```python
from build123d import *

# Parameters (mm, degrees)
SKETCH_1_R                  = 1.6
SKETCH_1_R_2                = 20
EXTRUDE_1_DEPTH             = 3
HOLE_WIZARD_M3_1_AT_2_COUNT = 2
HOLE_WIZARD_M3_1_AT_2_PITCH = 25
HOLE_WIZARD_M3_1_AT_3_COUNT = 2
HOLE_WIZARD_M3_1_AT_3_PITCH = 43.301270189
HOLE_WIZARD_M3_1_AT_4_COUNT = 2
HOLE_WIZARD_M3_1_AT_4_PITCH = 50
HOLE_WIZARD_M3_1_AT_5_COUNT = 2
HOLE_WIZARD_M3_1_AT_5_PITCH = 43.301270189
HOLE_WIZARD_M3_1_AT_6_COUNT = 2
HOLE_WIZARD_M3_1_AT_6_PITCH = 25
SKETCH_3_R                  = 1.6
CUT_EXTRUDE_1_DEPTH         = 10
CUT_EXTRUDE_2_DEPTH         = 10
FILLET_1_R                  = 2


with BuildPart() as part:
    # 草图1 → 凸台-拉伸1 (new body)
    with BuildSketch(Plane(origin=(0, 0, 0), x_dir=(1, 0, 0), z_dir=(0, 1, 0))):
        with BuildLine():
            Line((-63.2, 35), (0, 35))
            Line((0, 35), (0, -35))
            Line((0, -35), (-63.2, -35))
            ThreePointArc((-63.2, -35), (-98.2, 0), (-63.2, 35))
        make_face()
        with Locations(Location((-63.2, 25, 0), (0, 0, 270))):
            Circle(SKETCH_1_R, mode=Mode.SUBTRACT)
        with Locations(Location((-41.549364905, 12.5, 0), (0, 0, 270))):
            Circle(SKETCH_1_R, mode=Mode.SUBTRACT)
        with Locations(Location((-41.549364905, -12.5, 0), (0, 0, 270))):
            Circle(SKETCH_1_R, mode=Mode.SUBTRACT)
        with Locations(Location((-63.2, -25, 0), (0, 0, 270))):
            Circle(SKETCH_1_R, mode=Mode.SUBTRACT)
        with Locations(Location((-84.850635095, -12.5, 0), (0, 0, 270))):
            Circle(SKETCH_1_R, mode=Mode.SUBTRACT)
        with Locations(Location((-84.850635095, 12.5, 0), (0, 0, 270))):
            Circle(SKETCH_1_R, mode=Mode.SUBTRACT)
        with Locations(Location((-63.2, 0, 0), (0, 0, 270))):
            Circle(SKETCH_1_R_2, mode=Mode.SUBTRACT)
        with Locations(Location((-25, 20, 0), (0, 0, 270))):
            Circle(SKETCH_1_R, mode=Mode.SUBTRACT)
        with Locations(Location((-5, 20, 0), (0, 0, 270))):
            Circle(SKETCH_1_R, mode=Mode.SUBTRACT)
        with Locations(Location((-5, -20, 0), (0, 0, 270))):
            Circle(SKETCH_1_R, mode=Mode.SUBTRACT)
        with Locations(Location((-25, -20, 0), (0, 0, 270))):
            Circle(SKETCH_1_R, mode=Mode.SUBTRACT)
    extrude(amount=EXTRUDE_1_DEPTH)

    # 草图2 → M3 六角凹锥坑螺钉的锥形沉头孔1 (revolve, cut)
    with BuildSketch(Plane(origin=(-63.2, 3, -25), x_dir=(0, 0, 1), z_dir=(1, 0, 0))):
        Polygon((0, 0), (0, 3), (1.6, 3), (1.6, 1.76), (3.36, 0), align=None)
    hole_wizard_m3_1 = revolve(axis=Axis((-63.2, 9.35, -25), (0, -1, 0)), mode=Mode.SUBTRACT)

    # M3 六角凹锥坑螺钉的锥形沉头孔1 at 2: M3 六角凹锥坑螺钉的锥形沉头孔1 ×2
    with Locations(*[Vector(0.8660254037844387, 0, 0.5) * (i * HOLE_WIZARD_M3_1_AT_2_PITCH) for i in range(1, HOLE_WIZARD_M3_1_AT_2_COUNT)]):
        add(hole_wizard_m3_1, mode=Mode.SUBTRACT)

    # M3 六角凹锥坑螺钉的锥形沉头孔1 at 3: M3 六角凹锥坑螺钉的锥形沉头孔1 ×2
    with Locations(*[Vector(0.5000000000000001, 0, 0.8660254037844386) * (i * HOLE_WIZARD_M3_1_AT_3_PITCH) for i in range(1, HOLE_WIZARD_M3_1_AT_3_COUNT)]):
        add(hole_wizard_m3_1, mode=Mode.SUBTRACT)

    # M3 六角凹锥坑螺钉的锥形沉头孔1 at 4: M3 六角凹锥坑螺钉的锥形沉头孔1 ×2
    with Locations(*[(0, 0, i * HOLE_WIZARD_M3_1_AT_4_PITCH) for i in range(1, HOLE_WIZARD_M3_1_AT_4_COUNT)]):
        add(hole_wizard_m3_1, mode=Mode.SUBTRACT)

    # M3 六角凹锥坑螺钉的锥形沉头孔1 at 5: M3 六角凹锥坑螺钉的锥形沉头孔1 ×2
    with Locations(*[Vector(-0.49999999999999983, 0, 0.8660254037844388) * (i * HOLE_WIZARD_M3_1_AT_5_PITCH) for i in range(1, HOLE_WIZARD_M3_1_AT_5_COUNT)]):
        add(hole_wizard_m3_1, mode=Mode.SUBTRACT)

    # M3 六角凹锥坑螺钉的锥形沉头孔1 at 6: M3 六角凹锥坑螺钉的锥形沉头孔1 ×2
    with Locations(*[Vector(-0.8660254037844388, 0, 0.4999999999999997) * (i * HOLE_WIZARD_M3_1_AT_6_PITCH) for i in range(1, HOLE_WIZARD_M3_1_AT_6_COUNT)]):
        add(hole_wizard_m3_1, mode=Mode.SUBTRACT)

    # 草图3 → 切除-拉伸1 (cut)
    with BuildSketch(Plane(origin=(0, 3, 0), x_dir=(1, 0, 0), z_dir=(0, 1, 0))):
        with Locations(Location((-31.7, 0, 0), (0, 0, 270))):
            Circle(SKETCH_3_R)
        with Locations(Location((-47.45, -27.279800219, 0), (0, 0, 270))):
            Circle(SKETCH_3_R)
        with Locations(Location((-78.95, -27.279800219, 0), (0, 0, 270))):
            Circle(SKETCH_3_R)
        with Locations(Location((-94.7, 0, 0), (0, 0, 270))):
            Circle(SKETCH_3_R)
        with Locations(Location((-78.95, 27.279800219, 0), (0, 0, 270))):
            Circle(SKETCH_3_R)
        with Locations(Location((-47.45, 27.279800219, 0), (0, 0, 270))):
            Circle(SKETCH_3_R)
    extrude(amount=-CUT_EXTRUDE_1_DEPTH, mode=Mode.SUBTRACT)

    # 草图4 → 切除-拉伸2 (cut)
    with BuildSketch(Plane(origin=(0, 3, 0), x_dir=(1, 0, 0), z_dir=(0, 1, 0))):
        Polygon((-23.5, 13.645898034), (-23.5, -13.645898034), (-16.677050983, 0), align=None)
        Polygon((-15, -3.354101966), (-22.572949017, -18.5), (-7.427050983, -18.5), align=None)
        Polygon((-7.427050983, 18.5), (-22.572949017, 18.5), (-15, 3.354101966), align=None)
        Polygon((-13.322949017, 0), (-6.5, -13.645898034), (-6.5, 13.645898034), align=None)
    extrude(amount=-CUT_EXTRUDE_2_DEPTH, mode=Mode.SUBTRACT)

    # 圆角1
    fillet_1_edges = [part.edges().sort_by_distance(p)[0] for p in [
        (-22.572949017, 1.5, 18.5),
        (-15, 1.5, 3.354101966),
        (-7.427050983, 1.5, 18.5),
        (-22.572949017, 1.5, -18.5),
        (-7.427050983, 1.5, -18.5),
        (-15, 1.5, -3.354101966),
        (-13.322949017, 1.5, 0),
        (-6.5, 1.5, -13.645898034),
        (-6.5, 1.5, 13.645898034),
        (-23.5, 1.5, 13.645898034),
        (-23.5, 1.5, -13.645898034),
        (-16.677050983, 1.5, 0),
        (0, 1.5, -35),
        (0, 1.5, 35),
    ]]
    fillet(fillet_1_edges, radius=FILLET_1_R)


solid = part.part
```
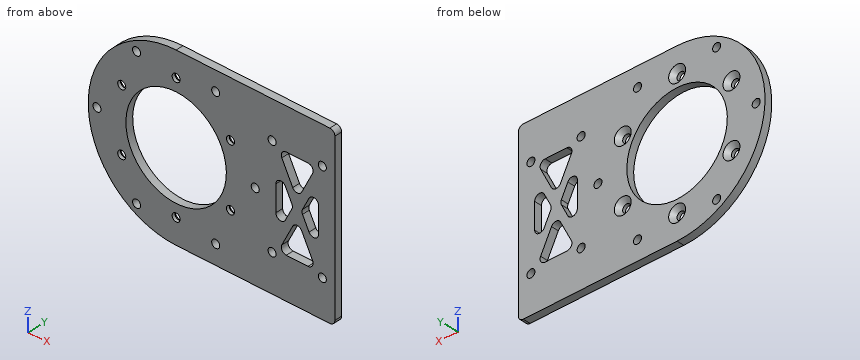
Check sheet for the modelled part. Datum: model origin and axes. Units: mm. Give positions to 0.01 mm unless a question says otherwise; leave off trailing zeros. Order: outer loops, then holes, each group sorted by start corner. A loop starts at its lowest first (then second) coordinate and runs counter-clockwise, first axis right, second up. Notation, with made-up numbers: (71, 17) -> (98, 17) arc R22 cw to (98, 47) -> close; hole circle Ø5 at (-32, -36). An arc over 180 degrees is marked (long way). Return JSON: item names as keys, results as strings.
1. Cross-section at B-B, the plane z = -17. Record the cut outline in (x, y).
From the geometry:
{"outline": "(-93.79, 0) -> (-73.74, 0) -> (-73.74, 3) -> (-93.79, 3) -> close; (-52.66, 0) -> (-21.27, 0) -> (-21.27, 3) -> (-52.66, 3) -> close; (-8.73, 0) -> (0, 0) -> (0, 3) -> (-8.73, 3) -> close"}
2. Material ranges on probe 1 along X at (y, z) = (2.4, 0); probe 2 along X at (y, z) = (2.8, 17); probe 3 along Z at (x, y) = (-14, 2.4), recorded low to high. Write a range as [from, to].
From the geometry:
{"probe 1": "[-98.2, -96.3], [-93.1, -83.2], [-43.2, -33.3], [-30.1, -23.5], [-16.91, -13.09], [-6.5, 0]", "probe 2": "[-93.79, -73.74], [-52.66, -21.27], [-8.73, 0]", "probe 3": "[-35, -18.5], [-6.09, 6.09], [18.5, 35]"}
3. Cross-section at C-C, the plane z = 12.5. Record the cut outline in (x, y), plus the area to 3 significant figures.
From the geometry:
{"outline": "(-95.89, 0) -> (-86.45, 0) -> (-86.45, 1.24) -> (-88.21, 3) -> (-95.89, 3) -> close; (-83.25, 0) -> (-78.81, 0) -> (-78.81, 3) -> (-81.49, 3) -> (-83.25, 1.24) -> close; (-47.59, 0) -> (-43.15, 0) -> (-43.15, 1.24) -> (-44.91, 3) -> (-47.59, 3) -> close; (-39.95, 0) -> (-19.57, 0) -> (-19.57, 3) -> (-38.19, 3) -> (-39.95, 1.24) -> close; (-10.43, 0) -> (0, 0) -> (0, 3) -> (-10.43, 3) -> close", "area": "141 mm^2"}
4. Cross-section at A-A, the plane x = -31.7. Record the cut outline in (y, z).
From the geometry:
{"outline": "(0, -35) -> (3, -35) -> (3, -1.6) -> (0, -1.6) -> close; (0, 1.6) -> (3, 1.6) -> (3, 35) -> (0, 35) -> close"}
5. Cross-section at D-D, the plane y = 2.3. Count the separate pieces of the cut face and the enclosed holes in it, plus the area to 3 significant figures.
From the geometry:
{"separate pieces": "1", "enclosed holes": "21", "area": "4,520 mm^2"}
